```python
from build123d import *

# Parameters (mm, degrees)
CENTRAL_POST_SKETCH_R       = 10
CENTRAL_POST_20_DEPTH       = 40
MOUNTING_PLATE_DEPTH        = 10
RECTANGULAR_PAD_60X30_DEPTH = 10
SIDE_WALL_SKETCH_W          = 10
SIDE_WALL_SKETCH_H          = 20
SIDE_WALL_DEPTH             = 30
HUB_SKETCH_R                = 15
HUB_30_DEPTH                = 10
PLATE_CUTOUTS_SKETCH_R      = 10
PLATE_CUTOUTS_DEPTH         = 10
SUPPORT_RIB_DEPTH           = 5
RIB_PATTERN_4X_COUNT        = 4


with BuildPart() as part:
    # Central Post Sketch → Central Post Ø20 (new, symmetric)
    with BuildSketch(Plane(origin=(0, 0, 0), x_dir=(1, 0, 0), z_dir=(0, 1, 0))):
        with Locations(Location((0, 0, 0), (0, 0, 270))):
            Circle(CENTRAL_POST_SKETCH_R)
    extrude(amount=CENTRAL_POST_20_DEPTH, both=True)

    # Plate Outline Sketch → Mounting Plate (add)
    with BuildSketch(Plane(origin=(0, 0, 0), x_dir=(1, 0, 0), z_dir=(0, 1, 0))):
        with BuildLine():
            Line((-65, 75), (0, 75))
            ThreePointArc((0, 75), (75, 0), (0, -75))
            Line((0, -75), (-65, -75))
            ThreePointArc((-65, -75), (-93.284271247, -63.284271247), (-105, -35))
            Line((-105, -35), (-105, 35))
            ThreePointArc((-105, 35), (-93.284271247, 63.284271247), (-65, 75))
        make_face()
    extrude(amount=-MOUNTING_PLATE_DEPTH)

    # Pad Sketch → Rectangular Pad 60x30 (add)
    with BuildSketch(Plane.XZ.offset(40)):
        with BuildLine():
            Line((-105, 30), (0, 30))
            ThreePointArc((0, 30), (30, 0), (0, -30))
            Line((0, -30), (-105, -30))
            Line((-105, -30), (-105, 30))
        make_face()
    extrude(amount=-RECTANGULAR_PAD_60X30_DEPTH)

    # Side Wall Sketch → Side Wall (add, symmetric)
    with BuildSketch(Plane.XY):
        with Locations((-100, -20)):
            Rectangle(SIDE_WALL_SKETCH_W, SIDE_WALL_SKETCH_H)
    extrude(amount=SIDE_WALL_DEPTH, both=True)

    # Hub Sketch → Hub Ø30 (add)
    with BuildSketch(Plane(origin=(0, 40, 0), x_dir=(1, 0, 0), z_dir=(0, 1, 0))):
        with Locations(Location((0, 0, 0), (0, 0, 270))):
            Circle(HUB_SKETCH_R)
    extrude(amount=-HUB_30_DEPTH)

    # Plate Cutouts Sketch → Plate Cutouts (cut)
    with BuildSketch(Plane(origin=(0, 0, 0), x_dir=(1, 0, 0), z_dir=(0, 1, 0))):
        with BuildLine():
            ThreePointArc((62.53594008, 17.727272727), (45.961940777, 45.961940777), (17.727272727, 62.53594008))
            ThreePointArc((17.727272727, 62.53594008), (8.969773108, 60.892266573), (5, 52.915026221))
            Line((5, 52.915026221), (5, 50))
            Line((5, 50), (-5, 50))
            Line((-5, 50), (-5, 55))
            ThreePointArc((-5, 55), (-7.928932188, 62.071067812), (-15, 65))
            Line((-15, 65), (-65, 65))
            ThreePointArc((-65, 65), (-95, 35), (-65, 5))
            Line((-65, 5), (-65, -5))
            ThreePointArc((-65, -5), (-95, -35), (-65, -65))
            Line((-65, -65), (-15, -65))
            ThreePointArc((-15, -65), (-7.928932188, -62.071067812), (-5, -55))
            Line((-5, -55), (-5, -50))
            Line((-5, -50), (5, -50))
            Line((5, -50), (5, -52.915026221))
            ThreePointArc((5, -52.915026221), (8.969773108, -60.892266573), (17.727272727, -62.53594008))
            ThreePointArc((17.727272727, -62.53594008), (45.961940777, -45.961940777), (62.53594008, -17.727272727))
            ThreePointArc((62.53594008, -17.727272727), (60.892266573, -8.969773108), (52.915026221, -5))
            Line((52.915026221, -5), (52.915026221, 5))
            ThreePointArc((52.915026221, 5), (60.892266573, 8.969773108), (62.53594008, 17.727272727))
        make_face()
        with Locations(Location((0, 0, 0), (0, 0, 270))):
            Circle(PLATE_CUTOUTS_SKETCH_R, mode=Mode.SUBTRACT)
    extrude(amount=-PLATE_CUTOUTS_DEPTH, mode=Mode.SUBTRACT)

    # Support Rib Sketch → Support Rib (add, symmetric)
    with BuildSketch(Plane.XY):
        with BuildLine():
            Line((0, 40), (-20, 40))
            ThreePointArc((-20, 40), (-30.606601718, 35.606601718), (-35, 25))
            Line((-35, 25), (-35, 15))
            ThreePointArc((-35, 15), (-39.393398282, 4.393398282), (-50, 0))
            Line((-50, 0), (-65, 0))
            Line((-65, 0), (-65, -10))
            Line((-65, -10), (-50, -10))
            ThreePointArc((-50, -10), (-32.32233047, -2.67766953), (-25, 15))
            Line((-25, 15), (-25, 25))
            ThreePointArc((-25, 25), (-23.535533906, 28.535533906), (-20, 30))
            Line((-20, 30), (0, 30))
            Line((0, 30), (0, 40))
        make_face()
    support_rib = extrude(amount=SUPPORT_RIB_DEPTH, both=True)

    # Rib Pattern 4x: Support Rib ×4 about axis
    rib_pattern_4x_axis = Axis((0, 0, 0), (0, 1, 0))
    for i in range(1, RIB_PATTERN_4X_COUNT):
        add(support_rib.rotate(rib_pattern_4x_axis, i * 360 / RIB_PATTERN_4X_COUNT))


solid = part.part
```
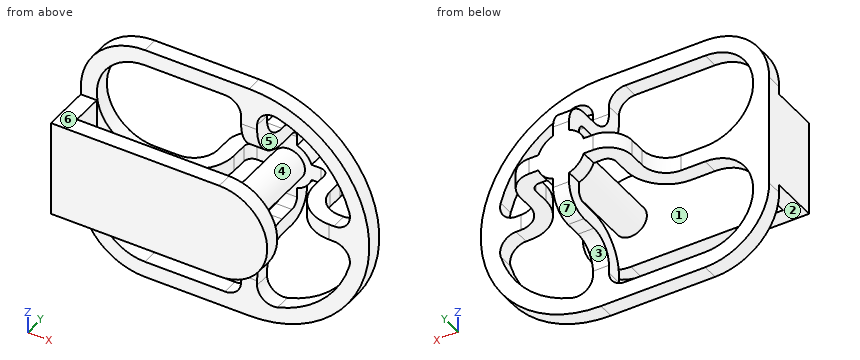
Read the model definition and answer for the solid it produces. Units are mm, in the model's axes. Face numbers are marked on the shaded views. A direction names the side the tool comes from. Give positions to 0.01 mm unless a question says otherwise; leave off trailing zeros. Loops run counter-clockwise (first coordinate to the right, second up) from the corner with the lowest first, then second, coordinate; pieces in that order, holes last.
Item 1: Each of these flat-tipped pins is pushed along its axis until it touches: pin 1 Ø8 at (y, z) = (-14.5, 42) entering from -X; pin 2 Ø19.5 at (x, y) = (30.5, 22.5) entering from -Z; pin 3 Ø5 at (y, z) = (19.5, -0.5) entering from -X; pin 4 Ø15 at (x, y) = (-39.5, 14.5) entering from +Z. Where does it stop, or does it pass through?
Item 2: The part is cut by section D-D (y = 27). Write down the section's boundary in (x, z).
Item 3: Find the intervals of material crossed by line 1 along Z through (x, y) = (-72.5, -1); line 2 along Z through (x, y) = (-33, 21); line 3 along X through (y, z) = (-10.5, -17), in increasing order.
Item 4: The part is cut by section C-C (x = 38.5). Write down the section's boundary in (y, z).
Item 5: The mould has two halves that part along Y. Classify the marked faces 1, 2, 3 and 4: released by +Y, released by -Y, zero draft, split by the parting line, or undercut.
Item 6: The part is cut by section B-B (z = 0). Write down the section's boundary in (x, y).
Item 7: The part is cut by section A-A (y = -4.5). Give the number of separate pieces and of enclosed holes in the cut face, and give its area (3 significant figures).
Item 8: For the marked faces 5, 6 and 7, determine the directions among +Z, -Z, +X, -X, +Y, -Y from which every point of the face is accessible in a straight line to the end or side of a thin tool.
Taken from the geometry:
1. pin 1: passes through
1. pin 2: stops at z = -5
1. pin 3: stops at x = -35
1. pin 4: stops at z = 5
2. outline: (-34.87, -5) - (-24.58, -5) - (-24.58, 5) - (-34.87, 5) - close; circle Ø20 at (0, 0); (-5, -34.87) - (5, -34.87) - (5, -24.58) - (-5, -24.58) - close; (-5, 24.58) - (5, 24.58) - (5, 34.87) - (-5, 34.87) - close; (24.58, -5) - (34.87, -5) - (34.87, 5) - (24.58, 5) - close
3. line 1: z = -74.29 to -64.05, -5.95 to 5.95, 64.05 to 74.29
3. line 2: z = -5 to 5
3. line 3: x = -105 to -95
4. outline: (-10, -64.36) - (0, -64.36) - (0, -52.37) - (-10, -52.37) - close; (-10, 52.37) - (0, 52.37) - (0, 64.36) - (-10, 64.36) - close; (-7.2, -5) - (5.37, -5) - (5.37, 5) - (-7.2, 5) - close
5. face 1: undercut
5. face 2: zero draft
5. face 3: released by +Y
5. face 4: undercut
6. outline: (-105, -40) - (30, -40) - (30, -30) - (10, -30) - (10, 30) - (20, 30) arc R5 cw to (25, 25) - (25, 15) arc R25 ccw to (50, -10) - (75, -10) - (75, 0) - (50, 0) arc R15 cw to (35, 15) - (35, 25) arc R15 ccw to (20, 40) - (-20, 40) arc R15 ccw to (-35, 25) - (-35, 15) arc R15 cw to (-50, 0) - (-105, 0) - close; hole (-95, -30) - (-10, -30) - (-10, 30) - (-20, 30) arc R5 ccw to (-25, 25) - (-25, 15) arc R25 cw to (-50, -10) - (-95, -10) - close
7. separate pieces: 2
7. enclosed holes: 1
7. area: 7,700 mm2
8. face 5: +Y
8. face 6: +Z, +X, -X, -Y
8. face 7: -Z, +X, -X, +Y
